Part model, mm, in its own coordinate system. Face numbers are marked on the shaded views. A direction names the side the tool comes from. Round coordinates to 2 decimals unless told otherwise and drop trailing zeros. Loops run counter-clockwise (first coordinate to the right, second up) from the corner with the lowest first, then second, coordinate; pieces in that order, holes last.
(1) Probe probe 1 along X at (y, z) = (15.5, -6.25); probe 2 along Z at (x, y) = (8.5, 49.5); probe 3 along Z at (x, y) = (7.25, 51). List the from-to ranges inside material, lowest first.
(2) Cut at A-A on y = 5. List the corners of the cut face in (x, z), then the cut area to 3 significant figures.
(3) Flat gauge pins, fed straight in: pin 1 (1 mm diameter, centred on y = 50, z = 5.5, fed in from +X); pin 2 (3 mm diameter, centred on x = 2, z = 4, fed in from +Y); pin 3 (5 mm diameter, centred on y = 48.5, z = -6.5, fed in from +X). Where does each tip first touch, or does it go through?
(4) Tool access for the marked faces 1 and 2: list every direction of +Z, -Z, +X, -X, +Y, -Y with a clear straight run to the whole face (end or side of a thin tool).
from build123d import *

# Parameters (mm, degrees)
SHANK_SKETCH_10_R          = 5
SHANK_10_DEPTH             = 11
SHANK_END_CHAMFER_0_5_SIZE = 0.5
COLLAR_SKETCH_16_R         = 8
COLLAR_16_DEPTH            = 8
COLLAR_FILLET_R2_R         = 2


with BuildPart() as part:
    # Shank Sketch Ø10 → Shank Ø10 (new body)
    with BuildSketch(Plane(origin=(0, 0, 0), x_dir=(1, 0, 0), z_dir=(0, 1, 0))):
        with Locations(Location((0, 0, 0), (0, 0, 270))):
            Circle(SHANK_SKETCH_10_R)
    extrude(amount=SHANK_10_DEPTH)

    # Shank End Chamfer 0.5
    shank_end_chamfer_0_5_edges = [part.edges().sort_by_distance(p)[0] for p in [
        (0, 0, -5),
    ]]
    chamfer(shank_end_chamfer_0_5_edges, length=SHANK_END_CHAMFER_0_5_SIZE)

    # Collar Sketch Ø16 → Collar Ø16 (add)
    with BuildSketch(Plane(origin=(0, 11, 0), x_dir=(1, 0, 0), z_dir=(0, 1, 0))):
        with Locations(Location((0, 0, 0), (0, 0, 270))):
            Circle(COLLAR_SKETCH_16_R)
    extrude(amount=COLLAR_16_DEPTH)

    # Collar Fillet R2
    collar_fillet_r2_edges = [part.edges().sort_by_distance(p)[0] for p in [
        (0, 11, -8),
    ]]
    fillet(collar_fillet_r2_edges, radius=COLLAR_FILLET_R2_R)

    # Grip Profile Sketch → Grip Knob (revolve)
    with BuildSketch(Plane.XY, mode=Mode.PRIVATE) as grip_knob_sk:
        with BuildLine():
            Line((-8, 19), (0, 19))
            Line((0, 19), (0, 72))
            ThreePointArc((0, 72), (-1.143202963, 71.811669668), (-2.165583383, 71.266582881))
            ThreePointArc((-2.165583383, 71.266582881), (-9.343191716, 55.495909404), (-5.86603911, 38.521174854))
            ThreePointArc((-5.86603911, 38.521174854), (-5.165533535, 28.567374361), (-8, 19))
        make_face()
    revolve(grip_knob_sk.sketch.rotate(Axis((0, 0, 0), (0, 1, 0)), 270), axis=Axis((0, 0, 0), (0, 1, 0)))


solid = part.part
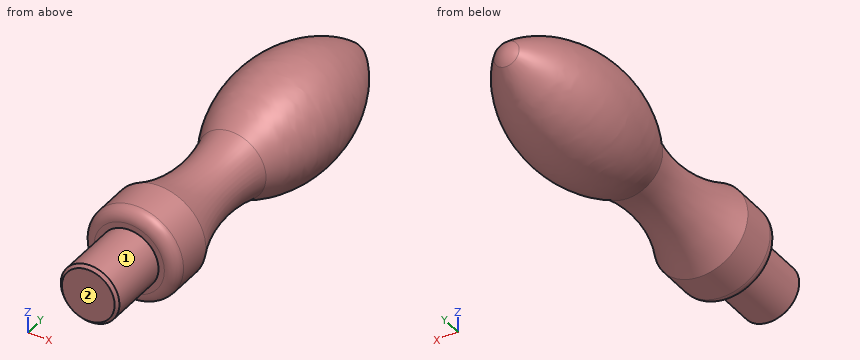
Final values:
1. probe 1: x = -4.99 to 4.99
1. probe 2: z = -3.95 to 3.95
1. probe 3: z = -6.12 to 6.12
2. outline: circle Ø10 at (0, 0)
2. area: 78.5 mm2
3. pin 1: stops at x = 7.99
3. pin 2: stops at y = 70.35
3. pin 3: stops at x = 8.4
4. face 1: -Y
4. face 2: +Z, -Z, +X, -X, -Y
